```python
from build123d import *

# Parameters (mm, degrees)
HEAT_SINK_BODY_EXTRUDE_80MM_DEPTH = 80


with BuildPart() as part:
    # Heat Sink Profile 20 Fins → Heat Sink Body Extrude 80mm (new body)
    with BuildSketch(Plane(origin=(0, 0, 0), x_dir=(1, 0, 0), z_dir=(0, 1, 0))):
        Polygon((-38.997486194, 17.547966284), (-39.997486194, 17.547966284), (-41.831758469, -17.452033716), (65.641252838, -17.452033716), (63.806980563, 17.547966284), (62.806980563, 17.547966284), (61.234747185, -12.452033716), (60.239213942, -12.452033716), (58.666980563, 17.547966284), (57.666980563, 17.547966284), (56.094747185, -12.452033716), (55.099213942, -12.452033716), (53.526980563, 17.547966284), (52.526980563, 17.547966284), (50.954747185, -12.452033716), (49.959213942, -12.452033716), (48.386980563, 17.547966284), (47.386980563, 17.547966284), (45.814747185, -12.452033716), (44.819213942, -12.452033716), (43.246980563, 17.547966284), (42.246980563, 17.547966284), (40.674747185, -12.452033716), (39.679213942, -12.452033716), (38.106980563, 17.547966284), (37.106980563, 17.547966284), (35.534747185, -12.452033716), (34.539213942, -12.452033716), (32.966980563, 17.547966284), (31.966980563, 17.547966284), (30.394747185, -12.452033716), (29.399213942, -12.452033716), (27.826980563, 17.547966284), (26.826980563, 17.547966284), (25.254747185, -12.452033716), (24.259213942, -12.452033716), (22.686980563, 17.547966284), (21.686980563, 17.547966284), (20.114747185, -12.452033716), (19.119213942, -12.452033716), (17.546980563, 17.547966284), (16.546980563, 17.547966284), (14.974747185, -12.452033716), (13.979213942, -12.452033716), (12.406980563, 17.547966284), (11.406980563, 17.547966284), (9.834747185, -12.452033716), (8.839213942, -12.452033716), (7.266980563, 17.547966284), (6.266980563, 17.547966284), (4.694747185, -12.452033716), (3.699213942, -12.452033716), (2.126980563, 17.547966284), (1.126980563, 17.547966284), (-0.445252815, -12.452033716), (-1.440786058, -12.452033716), (-3.013019437, 17.547966284), (-4.013019437, 17.547966284), (-5.585252815, -12.452033716), (-6.580786058, -12.452033716), (-8.153019437, 17.547966284), (-9.153019437, 17.547966284), (-10.725252815, -12.452033716), (-11.720786058, -12.452033716), (-13.293019437, 17.547966284), (-13.392304127, 17.547966284), (-14.293019437, 17.547966284), (-15.865252815, -12.452033716), (-16.860786058, -12.452033716), (-18.433019437, 17.547966284), (-19.433019437, 17.547966284), (-21.005252815, -12.452033716), (-22.000786058, -12.452033716), (-23.573019437, 17.547966284), (-24.573019437, 17.547966284), (-26.145252815, -12.452033716), (-27.140786058, -12.452033716), (-28.713019437, 17.547966284), (-29.713019437, 17.547966284), (-31.285252815, -12.452033716), (-32.280786058, -12.452033716), (-33.853019437, 17.547966284), (-34.853019437, 17.547966284), (-36.425252815, -12.452033716), (-37.425252815, -12.452033716), align=None)
    extrude(amount=HEAT_SINK_BODY_EXTRUDE_80MM_DEPTH)


solid = part.part
```
Work out the finished part from the listing and answer in its coordinate system (mm). Round coordinates to 2 decimals unless told otherwise and drop trailing zeros.
1) A cutting plane is placed at A-A on z = -14.5. Give the number of separate pieces and of enclosed holes in the cut face, and give its area (3 significant figures).
2) Determine the mould class of faces 1 (the face through (-9.93, 39.44, -2.76)), 2 (the face through (-40.9, 39.4, -0.3)) for opening direction X: pulls with the +X half, pulls with the -X half, needs draft (parallel to the pull), parting line crosses it, or undercut.
3) Consider probe 1 along Z at (x, y) = (-26.5, 39.5); probe 2 along X at (y, z) = (23, 13). Determine where each line is inside the solid, lowest interval first.
4) Flat-ended cylindrical pins translate along their axes: P1, Ø12, axis at y = 26.5, z = -1.5, coming from the +X side; P2, Ø0.8, axis at x = -21.5, y = 30, coming from the -Z side; P3, Ø2, axis at y = 66, z = -10.5, coming from the -X side. Find the tip coordinate at first contact, or state that the pin passes through.
Entries:
1. separate pieces: 21
1. enclosed holes: 0
1. area: 2,220 mm2
2. face 1: undercut
2. face 2: pulls with the -X half
3. probe 1: z = 12.45 to 17.45
3. probe 2: x = -41.6 to 65.41
4. P1: stops at x = 64.96
4. P2: stops at z = 12.45
4. P3: stops at x = -40.42
